Geometry check sheet. Reference: drawing and pictorial views, mm from the part's lowest x, y, z. Round coordinates to 2 decimals unless told otherwise and drop trailing zeros. Loops run counter-clockwise (first coordinate to the right, second up) from the corner with the lowest first, then second, coordinate; pieces in that order, holes last. Notation, with made-up numbers: (-21, 63) - (-6, 63) arc R31 cw to (-6, 97) - close; hole circle Ø3 at (74.5, -14). An arc over 180 degrees is marked (long way). Return JSON: item names as keys, results as strings.
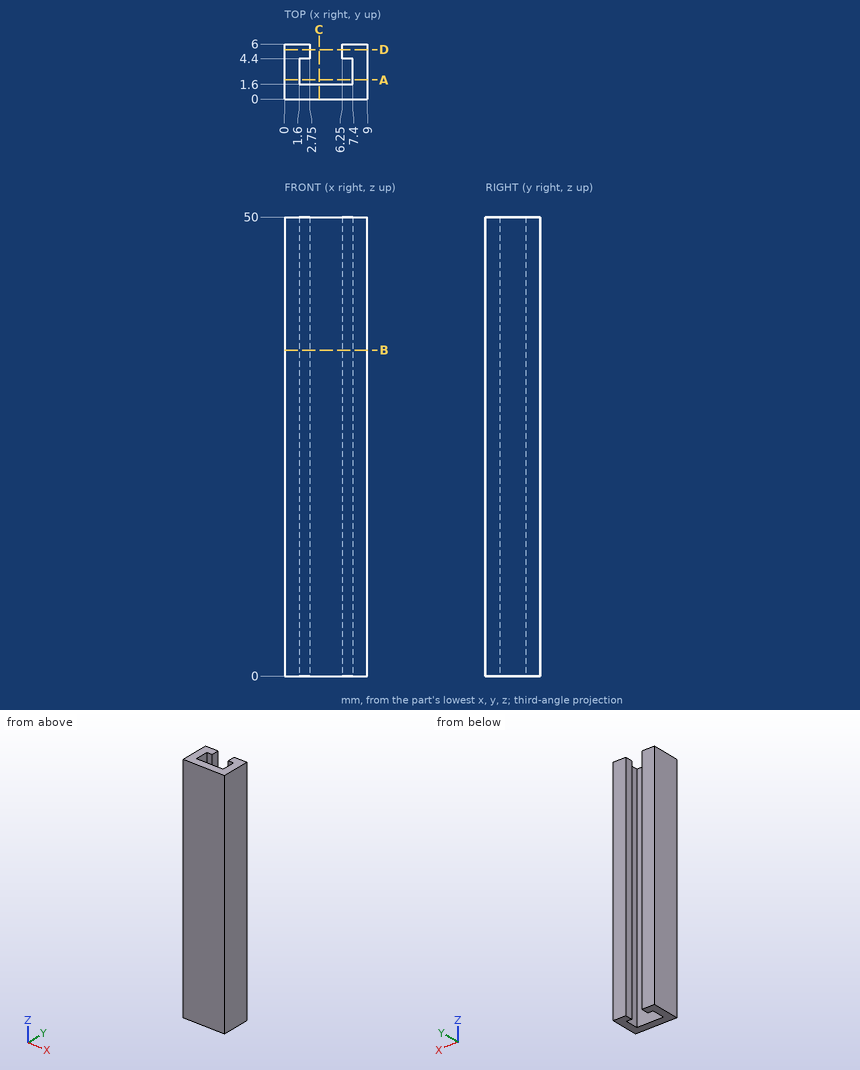
Q1. Sectioned sample at D-D (y = 5.4). Enter the section's corners in (x, z).
Answer key:
{"outline": "(0, 0) - (2.75, 0) - (2.75, 50) - (0, 50) - close; (6.25, 0) - (9, 0) - (9, 50) - (6.25, 50) - close"}
Q2. Depth check by flat-ended pin: P1, Ø1.5, axis at x = 6.5, z = 8.5, coming from the -Y side. Enter the tip coordinate at first touch or a pass-through.
Answer key:
{"P1": "stops at y = 0"}
Q3. Sectioned sample at B-B (z = 35.5). Enter the section's corners in (x, y).
Answer key:
{"outline": "(0, 0) - (9, 0) - (9, 6) - (6.25, 6) - (6.25, 4.4) - (7.4, 4.4) - (7.4, 1.6) - (1.6, 1.6) - (1.6, 4.4) - (2.75, 4.4) - (2.75, 6) - (0, 6) - close"}
Q4. Sectioned sample at C-C (x = 3.75). Enter the section's corners in (y, z).
Answer key:
{"outline": "(0, 0) - (1.6, 0) - (1.6, 50) - (0, 50) - close"}
Q5. Sectioned sample at A-A (y = 2.1). Enter the section's corners in (x, z).
Answer key:
{"outline": "(0, 0) - (1.6, 0) - (1.6, 50) - (0, 50) - close; (7.4, 0) - (9, 0) - (9, 50) - (7.4, 50) - close"}
Q6. Scan lines: probe 1 along X at (y, z) = (2.15, 42.5); probe 2 along Y at (x, z) = (7, 8.5); probe 3 along X at (y, z) = (5.75, 35). Record each from-to range of solid material in increasing order. Write a range as [from, to].
Answer key:
{"probe 1": "x = [0, 1.6], [7.4, 9]", "probe 2": "y = [0, 1.6], [4.4, 6]", "probe 3": "x = [0, 2.75], [6.25, 9]"}
